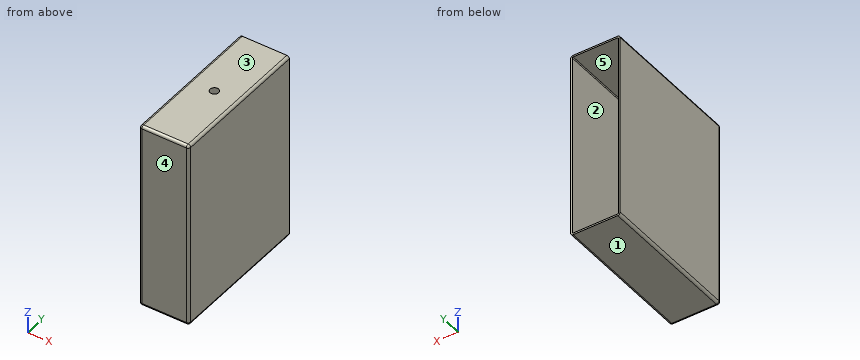
from build123d import *

# Parameters (mm, degrees)
SKETCH1_W             = 29
SKETCH1_H             = 110
BOSS_EXTRUDE1_DEPTH   = 42.5
FILLET1_R             = 1.5
SHELL1_T              = -1
SKETCH2_R             = 5
BOSS_EXTRUDE2_DEPTH   = 3
M6_TAPPED_HOLE1_D     = 5
M6_TAPPED_HOLE1_DEPTH = 4


with BuildPart() as part:
    # Sketch1 → Boss-Extrude1 (new, symmetric)
    with BuildSketch(Plane(origin=(0, 0, 0), x_dir=(1, 0, 0), z_dir=(0, 1, 0))):
        Rectangle(SKETCH1_W, SKETCH1_H)
    extrude(amount=BOSS_EXTRUDE1_DEPTH, both=True)

    # Fillet1
    fillet1_edges = [part.edges().sort_by_distance(p)[0] for p in [
        (0, -42.5, 55),
        (-14.5, -42.5, 0),
        (0, -42.5, -55),
        (14.5, -42.5, 0),
        (14.5, 0, 55),
        (-14.5, 0, 55),
        (-14.5, 0, -55),
        (14.5, 0, -55),
    ]]
    fillet(fillet1_edges, radius=FILLET1_R)

    # Shell1
    shell1_openings = [part.faces().sort_by_distance(p)[0] for p in [
        (0, 42.5, 0),
    ]]
    offset(amount=SHELL1_T, openings=shell1_openings, kind=Kind.INTERSECTION)

    # Sketch2 → Boss-Extrude2 (add)
    with BuildSketch(Plane(origin=(0, 0, 54), x_dir=(-1, 0, 0), z_dir=(0, 0, -1))):
        Circle(SKETCH2_R)
    extrude(amount=BOSS_EXTRUDE2_DEPTH)

    # M6 Tapped Hole1
    with Locations(Plane.XY.offset(55)):
        with Locations((0, 0)):
            Hole(M6_TAPPED_HOLE1_D / 2, depth=M6_TAPPED_HOLE1_DEPTH)


solid = part.part
For this review, take the finished solid that the model builds, in its own axes (mm). Face numbers are marked on the shaded views. A direction names the side the tool comes from. Round coordinates to 2 decimals unless told otherwise and drop trailing zeros. Loops run counter-clockwise (first coordinate to the right, second up) from the corner with the lowest first, then second, coordinate; pieces in that order, holes last. Notation, with made-up numbers: (48.25, 55) - (62.25, 55) arc R13 cw to (62.25, 69) - close; hole circle Ø10 at (-6.5, 65). An arc over 180 degrees is marked (long way). Use one line per item in the form item = value.
1) Tool access review of the marked faces 1 and 2: name each direction out of +Z, -Z, +X, -X, +Y, -Y from which nothing blocks a thin tool from reaching the whole face with its end or side.
Solutions:
face_1 = -Z, +X, -X, +Y, -Y
face_2 = +Y
2) We need section D-D on y = 0. Write out the cut boundary in (x, z).
Solutions:
outline = (-14.5, -53.5) arc R1.5 ccw to (-13, -55) - (13, -55) arc R1.5 ccw to (14.5, -53.5) - (14.5, 53.5) arc R1.5 ccw to (13, 55) - (2.5, 55) - (2.5, 51) - (5, 51) - (5, 54) - (13, 54) arc R0.5 cw to (13.5, 53.5) - (13.5, -53.5) arc R0.5 cw to (13, -54) - (-13, -54) arc R0.5 cw to (-13.5, -53.5) - (-13.5, 53.5) arc R0.5 cw to (-13, 54) - (-5, 54) - (-5, 51) - (-2.5, 51) - (-2.5, 55) - (-13, 55) arc R1.5 ccw to (-14.5, 53.5) - close
3) Wall thickness on probe 1 along Y at (x, z) = (0, 53.5); probe 2 along Z at (x, y) = (-11.25, 15); probe 3 along X at (y, z) = (19, 18): over which ranges is each line inside the solid? List them lowest first.
Solutions:
probe_1 = -42.5 to -41.5, -5 to -2.5, 2.5 to 5
probe_2 = -55 to -54, 54 to 55
probe_3 = -14.5 to -13.5, 13.5 to 14.5
4) We need section C-C on x = 9.5. Write out the cut boundary in (y, z).
Solutions:
outline = (-42.5, -53.5) arc R1.5 ccw to (-41, -55) - (42.5, -55) - (42.5, -54) - (-41, -54) arc R0.5 cw to (-41.5, -53.5) - (-41.5, 53.5) arc R0.5 cw to (-41, 54) - (42.5, 54) - (42.5, 55) - (-41, 55) arc R1.5 ccw to (-42.5, 53.5) - close
5) We need section B-B on x = 0. Write out the cut boundary in (y, z).
Solutions:
outline = (-42.5, -53.5) arc R1.5 ccw to (-41, -55) - (42.5, -55) - (42.5, -54) - (-41, -54) arc R0.5 cw to (-41.5, -53.5) - (-41.5, 53.5) arc R0.5 cw to (-41, 54) - (-5, 54) - (-5, 51) - (-2.5, 51) - (-2.5, 55) - (-41, 55) arc R1.5 ccw to (-42.5, 53.5) - close; (2.5, 51) - (5, 51) - (5, 54) - (42.5, 54) - (42.5, 55) - (2.5, 55) - close
6) Mouldability with a two-part tool opening along Y and no side actions: class the marked faces 3, 4 and 5 as pulls with the +Y half, pulls with the -Y half, needs draft (parallel to the pull), parting line crosses it, or undercut.
Solutions:
face_3 = needs draft
face_4 = pulls with the -Y half
face_5 = undercut
7) We need section A-A on y = -13. Write out the cut boundary in (x, z), then the cut area to 3 significant figures.
Solutions:
outline = (-14.5, -53.5) arc R1.5 ccw to (-13, -55) - (13, -55) arc R1.5 ccw to (14.5, -53.5) - (14.5, 53.5) arc R1.5 ccw to (13, 55) - (-13, 55) arc R1.5 ccw to (-14.5, 53.5) - close; hole (-13.5, -53.5) arc R0.5 ccw to (-13, -54) - (13, -54) arc R0.5 ccw to (13.5, -53.5) - (13.5, 53.5) arc R0.5 ccw to (13, 54) - (-13, 54) arc R0.5 ccw to (-13.5, 53.5) - close
area = 272 mm2
8) Clearance check with a flat-ended pin moving along its axis: P1, Ø3, axis at x = 4, z = 41.5, coming from the +Y side. State where the tip first meets the part, or that it passes through.
Solutions:
P1 = -41.5
